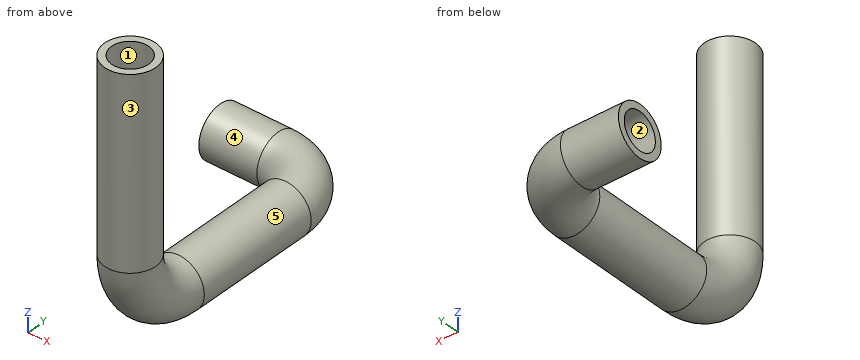
```python
from build123d import *

# Parameters (mm, degrees)
SKETCH_2_R   = 11
SKETCH_2_R_2 = 8
SKETCH_4_R   = 11
SKETCH_4_R_2 = 8


with BuildPart() as part:
    # Sweep 1: sweep along a path in Sketch 1
    with BuildLine(Plane.XY) as sweep_1_path:
        Line((0, 0), (25, 0))
        ThreePointArc((25, 0), (39.142135624, -5.857864376), (45, -20))
        Line((45, -20), (45, -50))
    # Sketch 2 → Sweep 1 (sweep)
    with BuildSketch(Plane(origin=(0, 0, 0), x_dir=(0, 0, -1), z_dir=(1, 0, 0))):
        Circle(SKETCH_2_R)
        Circle(SKETCH_2_R_2, mode=Mode.SUBTRACT)
    sweep(path=sweep_1_path.line)

    # Sweep 2: sweep along a path in Sketch 3
    with BuildLine(Plane(origin=(45, 0, 0), x_dir=(0, 0, -1), z_dir=(1, 0, 0))) as sweep_2_path:
        Line((0, -50), (0, -75))
        ThreePointArc((0, -75), (-7.32233047, -92.67766953), (-25, -100))
        Line((-25, -100), (-105.5, -100))
    # Sketch 4 → Sweep 2 (sweep)
    with BuildSketch(Plane.XZ.offset(50)):
        with Locations((45, 0)):
            Circle(SKETCH_4_R)
        with Locations((45, 0)):
            Circle(SKETCH_4_R_2, mode=Mode.SUBTRACT)
    sweep(path=sweep_2_path.line)


solid = part.part
```
The model under review builds one solid part; all positions refer to its coordinate system, in mm. Face numbers are marked on the shaded views. A direction names the side the tool comes from. Coordinates: 2 decimals unless noted, no trailing zeros. Write each loop counter-clockwise with the first axis right and the second up, starting at its lowest first coordinate (ties: lowest second). Pieces come first, ordered by that corner, then holes.
1) The part is to be moulded in two halves that separate along X. For the marked faces 1, 2 and 3, say which applies: pulls with the +X half, pulls with the -X half, needs draft (parallel to the pull), parting line crosses it, or undercut.
2) We need section B-B on y = -60.5. State the section outline as (x, z) points.
3) We need section A-A on x = 6. State the section outline as (y, z) points, then the cut area to 3 significant figures.
4) Clearance check with flat-ended pins moving along their axes: pin 1 Ø9.5 at (x, z) = (45, 0) entering from +Y; pin 2 Ø2 at (x, y) = (17, -3) entering from -Z; pin 3 Ø5 at (x, y) = (45.5, -1.5) entering from -Z; pin 4 Ø6 at (x, y) = (30.5, -47.5) entering from -Z. State where each tip first meets the part, or that it passes through.
5) Machinability: for the marked faces 4 and 5, which of the approach directions +Z, -Z, +X, -X, +Y, -Y give a long, thin tool a straight path to every point of the face, cutting with its end or side? Answer none if there is none.
6) To check wall thickness, follow probe 1 along Y at (x, z) = (45, 66); probe 2 along Y at (x, z) = (13, 0); probe 3 along X at (y, z) = (-52.5, 0). State the ranges of each line that lie inside material, in increasing order.
Answer list:
1. face 1: undercut
1. face 2: needs draft
1. face 3: parting line crosses it
2. outline: circle Ø22 at (45, 0); hole circle Ø16 at (45, 0)
3. outline: circle Ø22 at (0, 0); hole circle Ø16 at (0, 0)
3. area: 179 mm2
4. pin 1: stops at y = 6.99
4. pin 2: stops at z = -10.82
4. pin 3: stops at z = -9.74
4. pin 4: passes through
5. face 4: -X
5. face 5: none
6. probe 1: y = -111 to -108, -92 to -89
6. probe 2: y = -11 to -8, 8 to 11
6. probe 3: x = 34 to 37, 53 to 56
